Can you work these out from the model? Positions are in its coordinate system, mm. Face numbers are marked on the shaded views. Round coordinates to 2 decimals unless told otherwise and drop trailing zeros. Order: outer loops, then holes, each group sorted by start corner. A loop starts at its lowest first (then second) coordinate and runs counter-clockwise, first axis right, second up.
Q1. If we section it at C-C (z = -23): Please give me the cut outline in (x, y), plus the area to 3 significant figures.
Q2. Will these pins go through, and if not, where does the flat tip stop? P1, Ø1.8, axis at y = 11.5, z = 10, coming from the -X side; P2, Ø10, axis at y = 3, z = 20.5, coming from the +X side.
Q3. We'd pull the mould along Y, two halves only. Please class the marked faces 1, 2, 3 and 4: pulls with the +Y half, pulls with the -Y half, needs draft (parallel to the pull), parting line crosses it, or undercut.
Q4. If I drill on line 1 (Y direction, x = 1.45, z = 22.25); line 2 (Y direction, x = 4.8, z = 22.25); line 3 (X direction, y = -10, z = -28), over which ranges is the centre line in solid material (lowest first)?
Q5. If we section it at A-A (z = 10.25): Please give me the cut outline in (x, y), plus the area to 3 significant figures.
Q6. If we section it at B-B (x = 9): Please give me the cut outline in (y, z), plus the area to 3 significant figures.
Q7. If we section it at D-D (y = -6): Please give me the cut outline in (x, z).
from build123d import *

# Parameters (mm, degrees)
SKETCH1_W                                            = 60
SKETCH1_H                                            = 35
BOSS_EXTRUDE1_DEPTH                                  = 10
SKETCH2_W                                            = 60
SKETCH2_H                                            = 30
CUT_EXTRUDE1_DEPTH                                   = 2
CBORE_FOR_M3_HEXAGON_SOCKET_HEAD_CAP_SCR_D           = 3.4
CBORE_FOR_M3_HEXAGON_SOCKET_HEAD_CAP_SCR_CBORE_D     = 6
CBORE_FOR_M3_HEXAGON_SOCKET_HEAD_CAP_SCR_CBORE_DEPTH = 3.4
M4_TAPPED_HOLE1_D                                    = 3.3
M4_TAPPED_HOLE1_DEPTH                                = 10.1
M4_TAPPED_HOLE1_TIP                                  = 0.991420021


with BuildPart() as part:
    # Sketch1 → Boss-Extrude1 (new body)
    with BuildSketch(Plane(origin=(0, 0, 0), x_dir=(0, 0, -1), z_dir=(1, 0, 0))):
        Rectangle(SKETCH1_W, SKETCH1_H)
    extrude(amount=BOSS_EXTRUDE1_DEPTH)

    # Sketch2 → Cut-Extrude1 (cut)
    with BuildSketch(Plane(origin=(10, 0, 0), x_dir=(0, 0, -1), z_dir=(1, 0, 0))):
        Rectangle(SKETCH2_W, SKETCH2_H)
    extrude(amount=-CUT_EXTRUDE1_DEPTH, mode=Mode.SUBTRACT)

    # CBORE for M3 Hexagon socket head cap screws1 (through all)
    with Locations(Plane.ZY):
        with Locations((22.25, 10.5), (10.25, 10.5), (10.25, -10.5), (22.25, -10.5)):
            CounterBoreHole(CBORE_FOR_M3_HEXAGON_SOCKET_HEAD_CAP_SCR_D / 2, CBORE_FOR_M3_HEXAGON_SOCKET_HEAD_CAP_SCR_CBORE_D / 2, CBORE_FOR_M3_HEXAGON_SOCKET_HEAD_CAP_SCR_CBORE_DEPTH)

    # M4 Tapped Hole1
    with Locations(Plane(origin=(0, 0, -30), x_dir=(-1, 0, 0), z_dir=(0, 0, -1))):
        with Locations((-4, -10), (-4, 10)):
            Hole(M4_TAPPED_HOLE1_D / 2, depth=M4_TAPPED_HOLE1_DEPTH)
            with Locations((0, 0, -(M4_TAPPED_HOLE1_DEPTH + M4_TAPPED_HOLE1_TIP / 2))):  # 118° drill point
                Cone(0, M4_TAPPED_HOLE1_D / 2, M4_TAPPED_HOLE1_TIP, mode=Mode.SUBTRACT)


solid = part.part
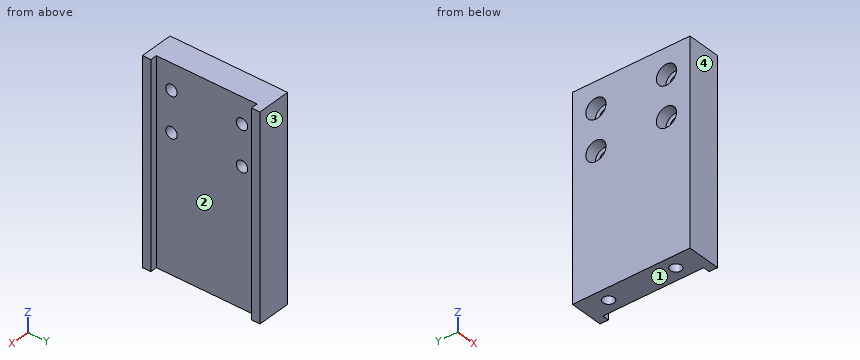
Solution:
1. outline: (0, -17.5) - (10, -17.5) - (10, -15) - (8, -15) - (8, 15) - (10, 15) - (10, 17.5) - (0, 17.5) - close; hole circle Ø3.3 at (4, -10); hole circle Ø3.3 at (4, 10)
1. area: 273 mm2
2. P1: stops at x = 3.4
2. P2: stops at x = 8
3. face 1: needs draft
3. face 2: undercut
3. face 3: pulls with the +Y half
3. face 4: pulls with the -Y half
4. line 1: y = -17.5 to -13.5, -7.5 to 7.5, 13.5 to 17.5
4. line 2: y = -17.5 to -12.2, -8.8 to 8.8, 12.2 to 17.5
4. line 3: x = 0 to 2.35, 5.65 to 8
5. outline: (0, -17.5) - (10, -17.5) - (10, -15) - (8, -15) - (8, -12.2) - (3.4, -12.2) - (3.4, -13.5) - (0, -13.5) - close; (0, -7.5) - (3.4, -7.5) - (3.4, -8.8) - (8, -8.8) - (8, 8.8) - (3.4, 8.8) - (3.4, 7.5) - (0, 7.5) - close; (0, 13.5) - (3.4, 13.5) - (3.4, 12.2) - (8, 12.2) - (8, 15) - (10, 15) - (10, 17.5) - (0, 17.5) - close
5. area: 218 mm2
6. outline: (-17.5, -30) - (-15, -30) - (-15, 30) - (-17.5, 30) - close; (15, -30) - (17.5, -30) - (17.5, 30) - (15, 30) - close
6. area: 300 mm2
7. outline: (0, -30) - (8, -30) - (8, 30) - (0, 30) - close
